```python
from build123d import *

# Parameters (mm, degrees)
EXTRUDE_1_DEPTH             = 115
EXTRUDE_START               = -10
EXTRUDE_2_DEPTH             = 10
EXTRUDE_START_2             = 10
EXTRUDE_3_DEPTH             = 10
SKETCH_4_R                  = 10.1
CUT_EXTRUDE_1_DEPTH         = 248.446964015
PATTERN_LINEAR_1_COUNT      = 2
PATTERN_LINEAR_1_PITCH      = 156
PATTERN_LINEAR_1_COUNT_DIR2 = 2
PATTERN_LINEAR_1_PITCH_DIR2 = 140


with BuildPart() as part:
    # 草图1 → 凸台-拉伸1 (new, symmetric)
    with BuildSketch(Plane.XY):
        Polygon((-143, 180), (-129, 180), (-129, 14), (129, 14), (129, 120), (143, 120), (143, 0), (-143, 0), align=None)
    extrude(amount=EXTRUDE_1_DEPTH, both=True)

    # 草图2 → 凸台-拉伸2 (add)
    with BuildSketch(Plane.XY.offset(EXTRUDE_START)):
        Polygon((129, 120), (129, 14), (-129, 14), (-129, 180), align=None)
    extrude(amount=-EXTRUDE_2_DEPTH)

    # 草图3 → 凸台-拉伸3 (add)
    with BuildSketch(Plane.XY.offset(EXTRUDE_START_2)):
        Polygon((-129, 180), (-129, 14), (129, 14), (129, 120), align=None)
    extrude(amount=EXTRUDE_3_DEPTH)

    # 草图4 → 切除-拉伸1 (cut, through all)
    with BuildSketch(Plane(origin=(0, 14, 0), x_dir=(1, 0, 0), z_dir=(0, 1, 0))):
        with Locations(Location((-74, -70, 0), (0, 0, 270))):
            Circle(SKETCH_4_R)
    cut_extrude_1 = extrude(amount=-CUT_EXTRUDE_1_DEPTH, mode=Mode.SUBTRACT)

    # 阵列(线性)1: Cut-Extrude 1 2 × 2
    with Locations(*[(i * PATTERN_LINEAR_1_PITCH, 0, -j * PATTERN_LINEAR_1_PITCH_DIR2) for i in range(PATTERN_LINEAR_1_COUNT) for j in range(PATTERN_LINEAR_1_COUNT_DIR2) if (i, j) != (0, 0)]):
        add(cut_extrude_1, mode=Mode.SUBTRACT)


solid = part.part
```
Check sheet for the modelled part. Datum: model origin and axes. Units: mm. A direction names the side the tool comes from. Coordinates: 2 decimals unless noted, no trailing zeros. Write each loop counter-clockwise with the first axis right and the second up, starting at its lowest first coordinate (ties: lowest second). Pieces come first, ordered by that corner, then holes. Notation, with made-up numbers: M 32.25,26 L 63.25,26 A19 ccw 63.25,59 Z; hole C 29,77.25 d4. An arc over 180 degrees is marked long. Write item = value, one per line. Start each with the question number.
1. Sectioned sample at C-C (x = 82). Record the cut outline in (y, z).
2. Sectioned sample at D-D (z = -38.5). Record the cut outline in (x, y), then the cut area to 3 significant figures.
3. Sectioned sample at B-B (y = 66). Record the cut outline in (x, z).
4. Tool access check on faces 5 (the flat face through (2, 80, -20)), 6 (the flat face through (-10, 10, 115)), 7 (the flat face through (-2, 14, 0)), 8 (the flat face through (129, 66, 68)). Record the directions out of +Z, -Z, +X, -X, +Y, -Y that give a thin tool (end or side, any length) a straight path to the whole face; none if there is none.
5. Mould release check, pull along X, two halves, no side actions. Record for faces 1 (the flat face through (129, 66, 0)), 2 (the flat face through (-2, 14, -67)), 3 (the flat face through (2, 0, 2)), 4 (the flat face through (-143, 89, 2)): pulls with the +X half, pulls with the -X half, needs draft (parallel to the pull), parting line crosses it, or undercut.
6. Sectioned sample at A-A (z = 70). Record the cut outline in (x, y).
7. Thickness scan on probe 1 along X at (y, z) = (7, 70); probe 2 along Z at (x, y) = (63, 98.5); probe 3 along X at (y, z) = (60.5, 24.5). Record the ranges inside material, lowest first.
8. Go/stop test with flat-tipped pins: pin 1 (2 mm diameter, centred on x = 99, y = 71.5, fed in from +Z); pin 2 (12 mm diameter, centred on x = -31.5, y = 134, fed in from -Z); pin 3 (23 mm diameter, centred on x = 82, z = -70, fed in from +Y); pin 4 (12 mm diameter, centred on x = 82, z = 70, fed in from +Y). Record where each tip stops, or that it passes through.
The answers:
q1.outline = M 0,-115 L 14,-115 L 14,-80.1 L 0,-80.1 Z; M 0,-59.9 L 14,-59.9 L 14,-20 L 130.93,-20 L 130.93,-10 L 14,-10 L 14,10 L 130.93,10 L 130.93,20 L 14,20 L 14,59.9 L 0,59.9 Z; M 0,80.1 L 14,80.1 L 14,115 L 0,115 Z
q2.outline = M -143,0 L 143,0 L 143,120 L 129,120 L 129,14 L -129,14 L -129,180 L -143,180 Z
q2.area = 7,810 mm²
q3.outline = M -143,-115 L -129,-115 L -129,-20 L 129,-20 L 129,-115 L 143,-115 L 143,115 L 129,115 L 129,20 L -129,20 L -129,115 L -143,115 Z; hole M -129,-10 L 129,-10 L 129,10 L -129,10 Z
q4.face_5 = -Z, +Y
q4.face_6 = +Z, +X, -X, +Y, -Y
q4.face_7 = +Y
q4.face_8 = +Z, +Y
q5.face_1 = undercut
q5.face_2 = undercut
q5.face_3 = needs draft
q5.face_4 = pulls with the -X half
q6.outline = M -143,0 L -84.1,0 L -84.1,14 L -129,14 L -129,180 L -143,180 Z; M -63.9,0 L 71.9,0 L 71.9,14 L -63.9,14 Z; M 92.1,0 L 143,0 L 143,120 L 129,120 L 129,14 L 92.1,14 Z
q7.probe_1 = -143 to -84.1, -63.9 to 71.9, 92.1 to 143
q7.probe_2 = -20 to -10, 10 to 20
q7.probe_3 = -143 to -129, 129 to 143
q8.pin_1 = 20
q8.pin_2 = -20
q8.pin_3 = 14
q8.pin_4 = through
